from build123d import *

# Parameters (mm, degrees)
SKETCH1_W               = 250
SKETCH1_H               = 20
BOSS_EXTRUDE1_DEPTH     = 365
CHAMFER1_SIZE           = 20
CUT_EXTRUDE1_DEPTH      = 443.860023032
CUT_EXTRUDE1_DEPTH_BACK = 443.860023032
SKETCH2_R               = 20
CHAMFER2_SIZE           = 20


with BuildPart() as part:
    # Sketch1 → Boss-Extrude1 (new body)
    with BuildSketch(Plane.XY):
        with Locations((-125, 10)):
            Rectangle(SKETCH1_W, SKETCH1_H)
    extrude(amount=BOSS_EXTRUDE1_DEPTH)

    # Chamfer1
    chamfer1_edges = [part.edges().sort_by_distance(p)[0] for p in [
        (-250, 10, 365),
    ]]
    chamfer(chamfer1_edges, length=CHAMFER1_SIZE)

    # Sketch2 → Cut-Extrude1 (cut, two sides: drawn at the far end of the back side and taken through both)
    with BuildSketch(Plane(origin=(0, 20, 0), x_dir=(1, 0, 0), z_dir=(0, 1, 0)).offset(-CUT_EXTRUDE1_DEPTH_BACK)):
        with Locations(Location((-200, -285, 0), (0, 0, 180))):
            Circle(SKETCH2_R)
    extrude(amount=CUT_EXTRUDE1_DEPTH + CUT_EXTRUDE1_DEPTH_BACK, mode=Mode.SUBTRACT)

    # Chamfer2
    chamfer2_edges = [part.edges().sort_by_distance(p)[0] for p in [
        (-250, 10, 0),
    ]]
    chamfer(chamfer2_edges, length=CHAMFER2_SIZE)


solid = part.part
Geometry: final body of the model. Coordinates: model frame, mm. Give positions to 0.01 mm unless a question says otherwise; leave off trailing zeros. Write each loop counter-clockwise with the first axis right and the second up, starting at its lowest first coordinate (ties: lowest second). Pieces come first, ordered by that corner, then holes. Notation, with made-up numbers: (50, 38) -> (92, 38) arc R28 cw to (92, 70) -> close; hole circle Ø6 at (-1.75, -13). An arc over 180 degrees is marked (long way). Answer as a JSON object with one key per item and string values.
1. Cut plane A-A on x = -200. Output: boundary loops of the cut face in (y, z).
Ans:
{"outline": "(0, 0) -> (20, 0) -> (20, 265) -> (0, 265) -> close; (0, 305) -> (20, 305) -> (20, 365) -> (0, 365) -> close"}
2. Mould query, pull axis Z, two halves, no side actions, for faces 1 (the flat face through (-240, 10, 10)), 2 (the cylindrical face through (-185.26, 9.86, 298.52)), 3 (the flat face through (0, 10, 180)). Classes: pulls with the +Z half, pulls with the -Z half, needs draft (parallel to the pull), parting line crosses it, or undercut.
Ans:
{"face 1": "pulls with the -Z half", "face 2": "undercut", "face 3": "needs draft"}
3. Contact query for a flat-ended pin moving along its axis: pin 1 (3 mm diameter, centred on y = 16.5, z = 320, fed in from +X). Output: stop coordinate, or through.
Ans:
{"pin 1": "stops at x = 0"}
4. Ray query, probe 1 along Z at (x, y) = (-200, 12.25); probe 2 along X at (y, z) = (5, 285); probe 3 along Z at (x, y) = (-209, 16.75). Return the intervals inside material, ascending. Write a range as from..to.
Ans:
{"probe 1": "z = 0..265, 305..365", "probe 2": "x = -250..-220, -180..0", "probe 3": "z = 0..267.14, 302.86..365"}
5. Cut plane C-C on z = 285. Output: boundary loops of the cut face in (x, y), and give its area (3 significant figures).
Ans:
{"outline": "(-250, 0) -> (-220, 0) -> (-220, 20) -> (-250, 20) -> close; (-180, 0) -> (0, 0) -> (0, 20) -> (-180, 20) -> close", "area": "4,200 mm^2"}
6. Cut plane B-B on y = 16.75. Output: boundary loops of the cut face in (x, z).
Ans:
{"outline": "(-250, 20) -> (-230, 0) -> (0, 0) -> (0, 365) -> (-230, 365) -> (-250, 345) -> close; hole circle Ø40 at (-200, 285)"}
